Source: CAD feature listing. Evaluate the final solid. Frame: model axes, mm. Face numbers are marked on the shaded views. A direction names the side the tool comes from. Coordinates: 2 decimals unless noted, no trailing zeros. Order: outer loops, then holes, each group sorted by start corner. A loop starts at its lowest first (then second) coordinate and runs counter-clockwise, first axis right, second up.
```python
from build123d import *

# Parameters (mm, degrees)
CRADLE_BLOCK_DEPTH      = 16
TAPERED_EXTENSION_DEPTH = 11
RELIEF_SLOT_PROFILE_W   = 12
RELIEF_SLOT_PROFILE_H   = 10
RELIEF_SLOT_DEPTH       = 52.378729511


with BuildPart() as part:
    # Cradle Block Profile → Cradle Block (new, symmetric)
    with BuildSketch(Plane.XY):
        with BuildLine():
            Line((11, 13), (16, 13))
            Line((16, 13), (16, -13))
            Line((16, -13), (-16, -13))
            Line((-16, -13), (-16, 13))
            Line((-16, 13), (-11, 13))
            ThreePointArc((-11, 13), (0, 2), (11, 13))
        make_face()
    extrude(amount=CRADLE_BLOCK_DEPTH, both=True)

    # Tapered Extension Profile → Tapered Extension (add, symmetric)
    with BuildSketch(Plane.XY):
        Polygon((-16, 13), (-28, 13), (-47, -4), (-47, -13), (-16, -13), align=None)
    extrude(amount=TAPERED_EXTENSION_DEPTH, both=True)

    # Relief Slot Profile → Relief Slot (cut, through all)
    with BuildSketch(Plane(origin=(-18.909230769, 21.133846154, 0), x_dir=(0.745241313525099, 0.6667948594698261, 0), z_dir=(-0.6667948594698261, 0.745241313525099, 0))):
        with Locations((-31.693521174, 0)):
            Rectangle(RELIEF_SLOT_PROFILE_W, RELIEF_SLOT_PROFILE_H)
    extrude(amount=-RELIEF_SLOT_DEPTH, mode=Mode.SUBTRACT)


solid = part.part
```
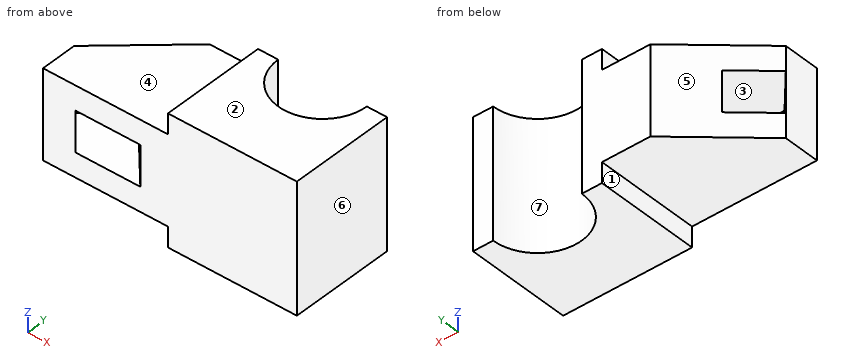
1. Access query for the marked faces 1, 2, 3 and 4. Directions: +Z, -Z, +X, -X, +Y, -Y. A direction counts if a zero-diameter tool reaches every point of the face in a straight line with its end or side. Return the directions, or none.
Findings:
face 1: -Z, -X, +Y, -Y
face 2: +Z, +X, -X, +Y, -Y
face 3: none
face 4: +Z, -X, +Y, -Y
2. Section query B-B on y = 3. Return loops of the section in (x, z).
Findings:
outline: (-39.18, -11) - (-16, -11) - (-16, -16) - (-4.58, -16) - (-4.58, 16) - (-16, 16) - (-16, 11) - (-39.18, 11) - (-39.18, 5) - (-37.16, 5) - (-37.16, -5) - (-39.18, -5) - close; (4.58, -16) - (16, -16) - (16, 16) - (4.58, 16) - close
3. Pin query (flat end, axial travel): P1, Ø4, axis at y = -5.5, z = -14, coming from the -X side; P2, Ø10, axis at x = -2, z = 5.5, coming from the +Y side; P3, Ø8, axis at x = -39, y = -6.5, coming from the +Z side. Return the tip coordinate at first contact, or that it passes through.
Findings:
P1: stops at x = -16
P2: stops at y = 4.51
P3: stops at z = 11
4. Ray query, line 1 (Y direction, x = 0.5, z = 0); line 2 (Z direction, x = -26.5, y = -1); line 3 (X direction, y = 7.25, z = 3). Return the intervals inside material, ascending.
Findings:
line 1: y = -13 to 2.01
line 2: z = -11 to 11
line 3: x = -34.43 to -9.38, 9.38 to 16
5. Section query D-D on y = -7.5. Return loops of the section in (x, z), plus the area to 3 significant figures.
Findings:
outline: (-47, -11) - (-16, -11) - (-16, -16) - (16, -16) - (16, 16) - (-16, 16) - (-16, 11) - (-47, 11) - close; hole (-43.87, -5) - (-27.77, -5) - (-27.77, 5) - (-43.87, 5) - close
area: 1,540 mm2
6. Section query C-C on z = 10. Return loops of the section in (x, y), plus the area to 3 significant figures.
Findings:
outline: (-47, -13) - (16, -13) - (16, 13) - (11, 13) arc R11 cw to (-11, 13) - (-28, 13) - (-47, -4) - close
area: 1,290 mm2
7. Draft query along X for the marked faces 5, 6 and 7. Return one class per face: released by +X, released by -X, zero draft, split by the parting line, or undercut.
Findings:
face 5: released by -X
face 6: released by +X
face 7: undercut
8. Section query A-A on z = -3.5. Return loops of the section in (x, y), plus the area to 3 significant figures.
Findings:
outline: (-47, -13) - (-38.95, -13) - (-47, -4) - close; (-38.06, 4) - (-22.85, -13) - (16, -13) - (16, 13) - (11, 13) arc R11 cw to (-11, 13) - (-28, 13) - close
area: 1,080 mm2
